The model under review builds one solid part; all positions refer to its coordinate system, in mm. Coordinates: 2 decimals unless noted, no trailing zeros. Write each loop counter-clockwise with the first axis right and the second up, starting at its lowest first coordinate (ties: lowest second). Pieces come first, ordered by that corner, then holes.
1) Add section B-B, the plane x = 0. State the section outline as (y, z) points.
2) For P1, Ø2.5, axis at x = 0, z = 33.34, coming from the +Y side; P2, Ø1, axis at y = 0, z = 6.5, coming from the -X side, all flat-tipped, find the tip position at first contact; note any pin that passes through.
3) Mouldability with a two-part tool opening along X and no side actions: class faces 1 (the cylindrical face through (31.874, 1.014, -0.325)), 2 (the flat face through (1, 0, 8)), 3 (the cylindrical face through (-39.05, 0.99, -8.67)) as released by +X, released by -X, zero draft, split by the parting line, or undercut.
4) Add section A-A, the plane z = 0. State the section outline as (x, y) points.
5) Add section D-D, the plane z = -18.5. State the section outline as (x, y) points.
6) Add section C-C, the plane y = 0.9. State the section outline as (x, z) points.
7) For line 1 (X direction, y = 1.35, z = 0); line 2 (Z direction, x = 31.5, y = 0.5); line 3 (Z direction, x = 25, y = 1.1), list the stretches that pass through material, from the lowest coordinate up.
from build123d import *

# Parameters (mm, degrees)
SKETCH1_R           = 40
BOSS_EXTRUDE1_DEPTH = 2
SKETCH2_R           = 3.5
CUT_EXTRUDE3_DEPTH  = 52
SKETCH3_R           = 1.5
CUT_EXTRUDE4_DEPTH  = 45


with BuildPart() as part:
    # Sketch1 → Boss-Extrude1 (new body)
    with BuildSketch(Plane(origin=(0, 0, 0), x_dir=(1, 0, 0), z_dir=(0, 1, 0))):
        with Locations(Location((0, 0, 0), (0, 0, 270))):
            Circle(SKETCH1_R)
    extrude(amount=BOSS_EXTRUDE1_DEPTH)

    # Sketch2 → Cut-Extrude3 (cut)
    with BuildSketch(Plane.XZ):
        with Locations(Location((0, 0, 0), (0, 0, 270))):
            Circle(SKETCH2_R)
    extrude(amount=-CUT_EXTRUDE3_DEPTH, mode=Mode.SUBTRACT)

    # Sketch3 → Cut-Extrude4 (cut)
    with BuildSketch(Plane(origin=(0, 2, 0), x_dir=(1, 0, 0), z_dir=(0, 1, 0))):
        with Locations(Location((0, 33.338700108, 0), (0, 0, 270))):
            Circle(SKETCH3_R)
        with Locations(Location((33.338700108, 0, 0), (0, 0, 270))):
            Circle(SKETCH3_R)
        with Locations(Location((0, -33.338700108, 0), (0, 0, 270))):
            Circle(SKETCH3_R)
        with Locations(Location((-33.338700108, 0, 0), (0, 0, 270))):
            Circle(SKETCH3_R)
    extrude(amount=-CUT_EXTRUDE4_DEPTH, mode=Mode.SUBTRACT)


solid = part.part
Geometry results:
1. outline: (0, -40) - (2, -40) - (2, -34.84) - (0, -34.84) - close; (0, -31.84) - (2, -31.84) - (2, -3.5) - (0, -3.5) - close; (0, 3.5) - (2, 3.5) - (2, 31.84) - (0, 31.84) - close; (0, 34.84) - (2, 34.84) - (2, 40) - (0, 40) - close
2. P1: passes through
2. P2: stops at x = -39.55
3. face 1: undercut
3. face 2: zero draft
3. face 3: split by the parting line
4. outline: (-40, 0) - (-34.84, 0) - (-34.84, 2) - (-40, 2) - close; (-31.84, 0) - (-3.5, 0) - (-3.5, 2) - (-31.84, 2) - close; (3.5, 0) - (31.84, 0) - (31.84, 2) - (3.5, 2) - close; (34.84, 0) - (40, 0) - (40, 2) - (34.84, 2) - close
5. outline: (-35.46, 0) - (35.46, 0) - (35.46, 2) - (-35.46, 2) - close
6. outline: circle Ø80 at (0, 0); hole circle Ø3 at (-33.34, 0); hole circle Ø7 at (0, 0); hole circle Ø3 at (0, -33.34); hole circle Ø3 at (0, 33.34); hole circle Ø3 at (33.34, 0)
7. line 1: x = -40 to -34.84, -31.84 to -3.5, 3.5 to 31.84, 34.84 to 40
7. line 2: z = -24.65 to 24.65
7. line 3: z = -31.22 to 31.22
